Geometry check sheet. Reference: the model listing, model coordinates, mm. A direction names the side the tool comes from. Round coordinates to 2 decimals unless told otherwise and drop trailing zeros. Order: outer loops, then holes, each group sorted by start corner. A loop starts at its lowest first (then second) coordinate and runs counter-clockwise, first axis right, second up. Notation, with made-up numbers: (58, 46) - (66, 46) arc R6 ccw to (66, 50) - close; hole circle Ø5 at (53.5, 55). An arc over 180 degrees is marked (long way). Return JSON: item names as keys, results as strings. Group by question number.
Q1. Sectioned sample at C-C, the plane x = -19. Record the cut outline in (y, z).
Q2. Material ranges on line 1 along X through (y, z) = (58, 12); line 2 along Z through (x, y) = (1.75, 8); line 3 along X through (y, z) = (8, 1.75), recorded low to high.
Q3. Gauge pin test, flat ends, axial feed: pin 1 Ø2 at (x, z) = (-5.5, 2) entering from +Y; pin 2 Ø4.5 at (x, z) = (18.5, 4) entering from -Y; pin 3 Ø5 at (y, z) = (73, 7.5) entering from -X; pin 4 Ø8 at (y, z) = (8, 7.52) entering from +X. Record the tip position at first contact, or that the pin passes through.
Q4. Sectioned sample at A-A, the plane y = 43. Record the cut outline in (x, z), then the cut area to 3 significant figures.
Q5. Tool access check on faces 1 (the flat face through (20, 58, 7)), 2 (the flat face through (-3, 15, 7)), 3 (the flat face through (2, 33, 0)), 4 (the flat face through (14, 30, 7)). Record the directions out of +Z, -Z, +X, -X, +Y, -Y that give a thin tool (end or side, any length) a straight path to the whole face; none if there is none.
Q6. Sectioned sample at D-D, the plane z = 1. Record the cut outline in (x, y).
Q7. Draft check along Z on faces 5 (the cylindrical face through (22.465, 70.139, 8.404)), 6 (the cylindrical face through (0, 0.5, 7.4)), 7 (the flat face through (-20, 57, 7)). Enter one of: pulls with the +Z half, pulls with the -Z half, needs draft (parallel to the pull), parting line crosses it, or undercut.
Q8. Sectioned sample at B-B, the plane z = 9. Record the cut outline in (x, y), then the cut area to 3 significant figures.
```python
from build123d import *

# Parameters (mm, degrees)
BOSS_EXTRUDE1_DEPTH = 15
SKETCH2_R           = 3
CUT_EXTRUDE1_DEPTH  = 100.749686716


with BuildPart() as part:
    # Sketch1 → Boss-Extrude1 (new body)
    with BuildSketch(Plane.XY):
        Polygon((20, 35), (-20, 35), (-20, 85), (-25, 85), (-25, 30), (-3, 30), (-3, 0), (0, 0), (3, 0), (3, 30), (25, 30), (25, 85), (20, 85), align=None)
    extrude(amount=BOSS_EXTRUDE1_DEPTH)

    # Sketch2 → Cut-Extrude1 (cut, through all)
    with BuildSketch(Plane.ZY.offset(25)):
        with Locations(Location((7.503230167, 72.999996799, 0), (0, 0, 270))):
            Circle(SKETCH2_R)
        with Locations(Location((7.523630467, 8, 0), (0, 0, 270))):
            Circle(SKETCH2_R)
        with BuildLine():
            Line((0.003230167, 72.999996799), (-23.0886588, 76.719933094))
            Line((-23.0886588, 76.719933094), (-0.661840838, 109.961720022))
            Line((-0.661840838, 109.961720022), (34.957913296, 90.556615978))
            Line((34.957913296, 90.556615978), (15.003230167, 72.999996799))
            ThreePointArc((15.003230167, 72.999996799), (7.503230167, 80.499996799), (0.003230167, 72.999996799))
        make_face()
        with BuildLine():
            Line((0.023630467, 8), (-15.301630232, 0.607134927))
            Line((-15.301630232, 0.607134927), (-3.280552195, -15.592363972))
            Line((-3.280552195, -15.592363972), (32.469088575, -12.351899457))
            Line((32.469088575, -12.351899457), (24.841547467, 4.357134927))
            Line((24.841547467, 4.357134927), (15.023630467, 8))
            ThreePointArc((15.023630467, 8), (7.523630467, 0.5), (0.023630467, 8))
        make_face()
    extrude(amount=-CUT_EXTRUDE1_DEPTH, mode=Mode.SUBTRACT)


solid = part.part
```
Reply:
{
 "1": {"outline": "(30, 0) - (35, 0) - (35, 15) - (30, 15) - close"},
 "2": {"line 1": "-25 to -20, 20 to 25", "line 2": "0 to 4.52, 10.52 to 15", "line 3": "-3 to 3"},
 "3": {"pin 1": "y = 35", "pin 2": "y = 30", "pin 3": "through", "pin 4": "x = 3"},
 "4": {"outline": "(-25, 0) - (-20, 0) - (-20, 15) - (-25, 15) - close; (20, 0) - (25, 0) - (25, 15) - (20, 15) - close", "area": "150 mm^2"},
 "5": {"face 1": "+Z, -Z, +Y", "face 2": "+Z, -Z, -X, -Y", "face 3": "-Z, +X, -X, +Y, -Y", "face 4": "+Z, -Z, +X, -Y"},
 "6": {"outline": "(-25, 30) - (-3, 30) - (-3, 4.3) - (3, 4.3) - (3, 30) - (25, 30) - (25, 76.74) - (20, 76.74) - (20, 35) - (-20, 35) - (-20, 76.74) - (-25, 76.74) - close"},
 "7": {"face 5": "undercut", "face 6": "parting line crosses it", "face 7": "needs draft"},
 "8": {"outline": "(-25, 30) - (-3, 30) - (-3, 10.61) - (3, 10.61) - (3, 30) - (25, 30) - (25, 70.4) - (20, 70.4) - (20, 35) - (-20, 35) - (-20, 70.4) - (-25, 70.4) - close; (-25, 75.6) - (-20, 75.6) - (-20, 80.35) - (-25, 80.35) - close; (-3, 0.65) - (3, 0.65) - (3, 5.39) - (-3, 5.39) - close; (20, 75.6) - (25, 75.6) - (25, 80.35) - (20, 80.35) - close", "area": "796 mm^2"}
}
